Work out the finished part from the listing and answer in its coordinate system (mm). A direction names the side the tool comes from. Round coordinates to 2 decimals unless told otherwise and drop trailing zeros. Write each loop counter-clockwise with the first axis right and the second up, starting at its lowest first coordinate (ties: lowest second). Pieces come first, ordered by that corner, then holes.
from build123d import *


with BuildPart() as part:
    # Sketch1 → Revolve1 (revolve)
    with BuildSketch(Plane.XY, mode=Mode.PRIVATE) as revolve1_sk:
        with BuildLine():
            Line((0, 3.42), (0, 3.2))
            Line((0, 3.2), (0.255, 3.2))
            Line((0.255, 3.2), (0.255, 2.575))
            Line((0.255, 2.575), (0, 2.575))
            Line((0, 2.575), (0, 2.08))
            ThreePointArc((0, 2.08), (0.023431458, 2.023431458), (0.08, 2))
            Line((0.08, 2), (2.42, 2))
            ThreePointArc((2.42, 2), (2.476568542, 2.023431458), (2.5, 2.08))
            Line((2.5, 2.08), (2.5, 2.575))
            Line((2.5, 2.575), (2.245, 2.575))
            Line((2.245, 2.575), (2.245, 3.2))
            Line((2.245, 3.2), (2.5, 3.2))
            Line((2.5, 3.2), (2.5, 3.42))
            ThreePointArc((2.5, 3.42), (2.476568542, 3.476568542), (2.42, 3.5))
            Line((2.42, 3.5), (0.08, 3.5))
            ThreePointArc((0.08, 3.5), (0.023431458, 3.476568542), (0, 3.42))
        make_face()
    revolve(revolve1_sk.sketch.rotate(Axis((2.42, 0, 0), (-1, 0, 0)), 270), axis=Axis((2.42, 0, 0), (-1, 0, 0)))


solid = part.part
Q1. Find the intervals of material crossed by L1, parallel to Y at x = 0.2, z = 0 (3 decimals); L2, parallel to X at y = 3, z = 0.25 (3 decimals); L3, parallel to Y at x = 1.05, z = 0, in increasing order.
Q2. Given pin 1 (3 mm diameter, centred on y = 1.5, z = -1.5, fed in from -X), flat-ended and moving along its own axis, determine where the tip first touches the part or whether it passes through.
Q3. Find section C-C (x = 1.5). Determine the outline of the cut face in (y, z), plus the area to 3 significant figures.
Q4. The mould has two halves that part along Z. Classify faces 3 (the face through (1.234, -3.417, -0.759)), 4 (the face through (0.255, 3, 0)), 5 (the face through (2.5, -2, -1)): +Z half, -Z half, draft (parallel to the pull), parting line (faces both ways), or undercut.
Q5. A tool of negligible diameter and unlimited length cuts with its end or side. For faces 1 (the face through (2.245, 3, 0)), 2 (the face through (0, -2, 1)), from which of +Z, -Z, +X, -X, +Y, -Y can it reach the whole face along a straight path? Write none if from no direction.
Report:
1. L1: y = -3.5 to -3.2, -2.575 to -2, 2 to 2.575, 3.2 to 3.5
1. L2: x = 0.255 to 2.245
1. L3: y = -3.5 to -2, 2 to 3.5
2. pin 1: stops at x = 0
3. outline: circle Ø7 at (0, 0); hole circle Ø4 at (0, 0)
3. area: 25.9 mm2
4. face 3: parting line
4. face 4: undercut
4. face 5: draft
5. face 1: +X
5. face 2: +Z, -Z, -X, +Y, -Y
